from build123d import *

# Parameters (mm, degrees)
EXTRUDE_1_DEPTH = 7


with BuildPart() as part:
    # 草图1 → 凸台-拉伸1 (new, symmetric)
    with BuildSketch(Plane.XY):
        Polygon((0, 0), (0, 85), (26, 85), (26, 40), (15, 0), align=None)
    extrude(amount=EXTRUDE_1_DEPTH, both=True)


solid = part.part
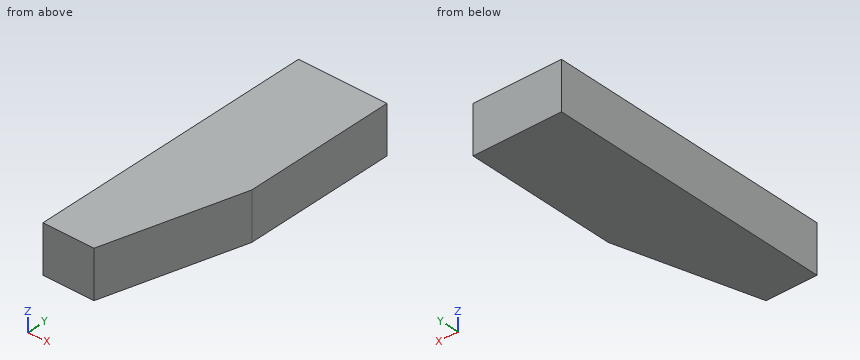
Check sheet for the modelled part. Datum: model origin and axes. Units: mm. Give positions to 0.01 mm unless a question says otherwise; leave off trailing zeros. Loops run counter-clockwise (first coordinate to the right, second up) from the corner with the lowest first, then second, coordinate; pieces in that order, holes last. Notation, with made-up numbers: M -12.75,23.5 L 11.25,23.5 A22 ccw 11.25,43.5 Z; hole C 71.5,30 d11. An arc over 180 degrees is marked long. Return JSON: item names as keys, results as strings. Group by question number.
1. Cross-section at B-B on y = 38. Record the boundary of the cut face in (x, z), plus the area to 3 significant figures.
2. Cross-section at C-C on x = 22.25. Record the boundary of the cut face in (y, z), plus the area to 3 significant figures.
3. Cross-section at A-A on z = 5.25. Record the boundary of the cut face in (x, y).
4. Thickness scan on L1, parallel to X at y = 4, z = 3; L2, parallel to X at y = 23.5, z = 4. Record the ranges inside material, lowest first.
Return value:
{
 "1": {"outline": "M 0,-7 L 25.45,-7 L 25.45,7 L 0,7 Z", "area": "356 mm^2"},
 "2": {"outline": "M 26.36,-7 L 85,-7 L 85,7 L 26.36,7 Z", "area": "821 mm^2"},
 "3": {"outline": "M 0,0 L 15,0 L 26,40 L 26,85 L 0,85 Z"},
 "4": {"L1": "0 to 16.1", "L2": "0 to 21.46"}
}
